Check sheet for the modelled part. Datum: model origin and axes. Units: mm. Face numbers are marked on the shaded views. Coordinates: 2 decimals unless noted, no trailing zeros. Loops run counter-clockwise (first coordinate to the right, second up) from the corner with the lowest first, then second, coordinate; pieces in that order, holes last. Notation, with made-up numbers: (7, 47.25) -> (55, 47.25) arc R11 ccw to (55, 59.25) -> close; hole circle Ø6 at (1.25, 16.5). An arc over 180 degrees is marked (long way). Use one line per item in the form item = value.
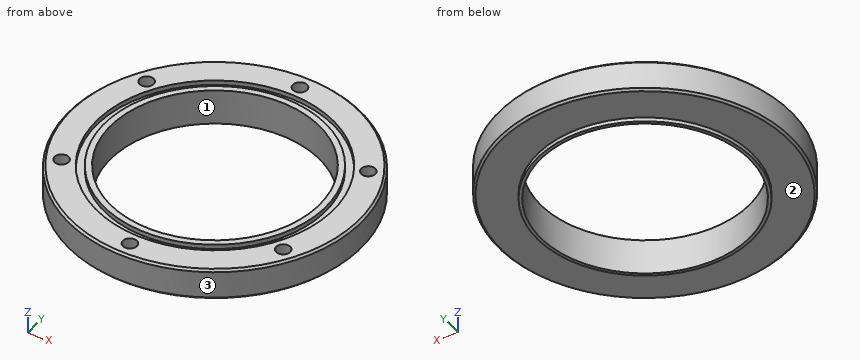
from build123d import *

# Parameters (mm, degrees)
SKETCH1_R             = 70
SKETCH1_R_2           = 50
BOSS_EXTRUDE1_DEPTH   = 17
SKETCH2_R             = 56.65
SKETCH2_R_2           = 52.95
CUT_EXTRUDE1_DEPTH    = 2.2
SKETCH3_R             = 70
SKETCH3_R_2           = 51.5
CUT_EXTRUDE2_DEPTH    = 2
SKETCH4_R             = 3
CUT_EXTRUDE3_DEPTH    = 10
M8_TAPPED_HOLE1_D     = 6.8
M8_TAPPED_HOLE1_DEPTH = 10
M8_TAPPED_HOLE1_TIP   = 2.042926105
CHAMFER1_SIZE         = 1


with BuildPart() as part:
    # Sketch1 → Boss-Extrude1 (new body)
    with BuildSketch(Plane.XY):
        Circle(SKETCH1_R)
        Circle(SKETCH1_R_2, mode=Mode.SUBTRACT)
    extrude(amount=BOSS_EXTRUDE1_DEPTH)

    # Sketch2 → Cut-Extrude1 (cut)
    with BuildSketch(Plane.XY.offset(17)):
        Circle(SKETCH2_R)
        Circle(SKETCH2_R_2, mode=Mode.SUBTRACT)
    extrude(amount=-CUT_EXTRUDE1_DEPTH, mode=Mode.SUBTRACT)

    # Sketch3 → Cut-Extrude2 (cut)
    with BuildSketch(Plane(origin=(0, 0, 0), x_dir=(-1, 0, 0), z_dir=(0, 0, -1))):
        Circle(SKETCH3_R)
        Circle(SKETCH3_R_2, mode=Mode.SUBTRACT)
    extrude(amount=-CUT_EXTRUDE2_DEPTH, mode=Mode.SUBTRACT)

    # Sketch4 → Cut-Extrude3 (cut)
    with BuildSketch(Plane.XY.offset(17)):
        with Locations((0, 62.5)):
            Circle(SKETCH4_R)
        with Locations((54.126587737, 31.25)):
            Circle(SKETCH4_R)
        with Locations((54.126587737, -31.25)):
            Circle(SKETCH4_R)
        with Locations((0, -62.5)):
            Circle(SKETCH4_R)
        with Locations((-54.126587737, -31.25)):
            Circle(SKETCH4_R)
        with Locations((-54.126587737, 31.25)):
            Circle(SKETCH4_R)
    extrude(amount=-CUT_EXTRUDE3_DEPTH, mode=Mode.SUBTRACT)

    # M8 Tapped Hole1
    with Locations(Plane.XY.offset(17)):
        with Locations((0, 62.5), (54.126587737, 31.25), (54.126587737, -31.25), (0, -62.5), (-54.126587737, -31.25), (-54.126587737, 31.25)):
            Hole(M8_TAPPED_HOLE1_D / 2, depth=M8_TAPPED_HOLE1_DEPTH)
            with Locations((0, 0, -(M8_TAPPED_HOLE1_DEPTH + M8_TAPPED_HOLE1_TIP / 2))):  # 118° drill point
                Cone(0, M8_TAPPED_HOLE1_D / 2, M8_TAPPED_HOLE1_TIP, mode=Mode.SUBTRACT)

    # Chamfer1
    chamfer1_edges = [part.edges().sort_by_distance(p)[0] for p in [
        (-70, 0, 2),
        (-70, 0, 17),
    ]]
    chamfer(chamfer1_edges, length=CHAMFER1_SIZE)


solid = part.part
(1) Scan lines: line 1 along Y through (x, z) = (0, 13.5); line 2 along X through (y, z) = (-45, 15.5); line 3 along X through (y, z) = (31.25, 9.75). Record each from-to range of solid material in increasing order.
Established:
line_1 = -70 to -65.9, -59.1 to -50, 50 to 59.1, 65.9 to 70
line_2 = -53.62 to -34.41, -27.91 to -21.79, 21.79 to 27.91, 34.41 to 53.62
line_3 = -62.64 to -57.53, -50.73 to -39.03, 39.03 to 50.73, 57.53 to 62.64
(2) Go/stop test with flat-tipped pins: P1, Ø10, axis at y = 19.5, z = 6, coming from the +X side; P2, Ø6, axis at y = 20, z = 13, coming from the -X side; P3, Ø1.5, axis at x = 23.5, z = 8, coming from the +Y side. Record where each tip stops, or that it passes through.
Established:
P1 = 68.48
P2 = -67.9
P3 = 66.2
(3) Section check A-A, the plane y = 0. Record the boundary of the cut face in (x, z), plus the area to 3 significant figures.
Established:
outline = (-70, 3) -> (-69, 2) -> (-51.5, 2) -> (-51.5, 0) -> (-50, 0) -> (-50, 17) -> (-52.95, 17) -> (-52.95, 14.8) -> (-56.65, 14.8) -> (-56.65, 17) -> (-69, 17) -> (-70, 16) -> close; (50, 0) -> (51.5, 0) -> (51.5, 2) -> (69, 2) -> (70, 3) -> (70, 16) -> (69, 17) -> (56.65, 17) -> (56.65, 14.8) -> (52.95, 14.8) -> (52.95, 17) -> (50, 17) -> close
area = 588 mm²
(4) Section check B-B, the plane z = 13. Record the boundary of the cut face in (x, y), plus the area to 3 significant figures.
Established:
outline = circle Ø140 at (0, 0); hole circle Ø6.8 at (-54.13, -31.25); hole circle Ø6.8 at (-54.13, 31.25); hole circle Ø100 at (0, 0); hole circle Ø6.8 at (0, -62.5); hole circle Ø6.8 at (0, 62.5); hole circle Ø6.8 at (54.13, -31.25); hole circle Ø6.8 at (54.13, 31.25)
area = 7,320 mm²
(5) Mould release check, pull along X, two halves, no side actions. Record for the marked faces 1, 2 and 3: +X half, -X half, draft (parallel to the pull), parting line (faces both ways), or undercut.
Established:
face_1 = undercut
face_2 = draft
face_3 = parting line
